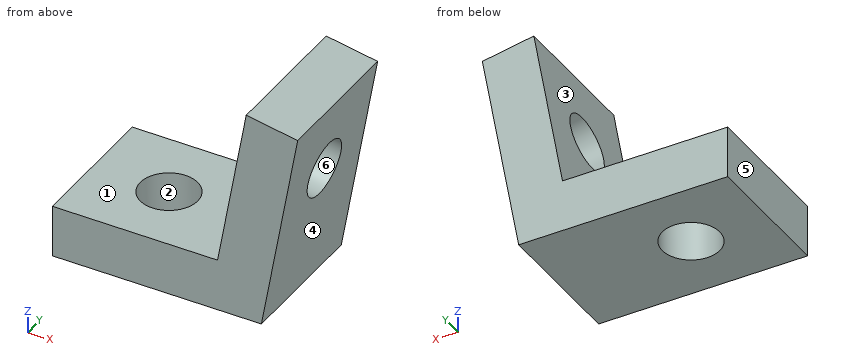
```python
from build123d import *

# Parameters (mm, degrees)
SKETCH_1_W          = 12
SKETCH_1_H          = 8
EXTRUDE_1_DEPTH     = 3
EXTRUDE_2_DEPTH     = 8
SKETCH_3_R          = 1.65
CUT_EXTRUDE_1_DEPTH = 3
SKETCH_4_R          = 1.65
CUT_EXTRUDE_2_DEPTH = 3


with BuildPart() as part:
    # 草图1 → 凸台-拉伸1 (new body)
    with BuildSketch(Plane.XY):
        with Locations((-1.4, 0)):
            Rectangle(SKETCH_1_W, SKETCH_1_H)
    extrude(amount=EXTRUDE_1_DEPTH)

    # 草图2 → 凸台-拉伸2 (add)
    with BuildSketch(Plane.XZ.offset(4)):
        Polygon((4.6, 0), (6.683778132, 11.817693036), (3.729354873, 12.338637569), (2.082701106, 3), align=None)
    extrude(amount=-EXTRUDE_2_DEPTH)

    # 草图3 → 切除-拉伸1 (cut)
    with BuildSketch(Plane.XY.offset(3)):
        with Locations((-3, 0)):
            Circle(SKETCH_3_R)
    extrude(amount=-CUT_EXTRUDE_1_DEPTH, mode=Mode.SUBTRACT)

    # 草图4 → 切除-拉伸2 (cut)
    with BuildSketch(Plane(origin=(4.461293028, 0, -0.78664633), x_dir=(-0.1736481776669236, 0, -0.9848077530122092), z_dir=(0.9848077530122092, 0, -0.1736481776669236))):
        with Locations((-8.398781617, 0)):
            Circle(SKETCH_4_R)
    extrude(amount=-CUT_EXTRUDE_2_DEPTH, mode=Mode.SUBTRACT)


solid = part.part
```
Work out the finished part from the listing and answer in its coordinate system (mm). Face numbers are marked on the shaded views. A direction names the side the tool comes from. Give positions to 0.01 mm unless a question says otherwise; leave off trailing zeros. Order: outer loops, then holes, each group sorted by start corner. A loop starts at its lowest first (then second) coordinate and runs counter-clockwise, first axis right, second up.
1. Section B-B, the plane y = -1.25 is taken. Determine the outline of the cut face in (x, z).
Result sheet:
outline: (-7.4, 0) - (-4.08, 0) - (-4.08, 3) - (-7.4, 3) - close; (-1.92, 0) - (4.6, 0) - (5.73, 6.42) - (2.78, 6.94) - (2.08, 3) - (-1.92, 3) - close; (3.15, 9.07) - (6.11, 8.55) - (6.68, 11.82) - (3.73, 12.34) - close
2. Section A-A, the plane x = -3 is taken. Determine the outline of the cut face in (y, z), and give its area (3 significant figures).
Result sheet:
outline: (-4, 0) - (-1.65, 0) - (-1.65, 3) - (-4, 3) - close; (1.65, 0) - (4, 0) - (4, 3) - (1.65, 3) - close
area: 14.1 mm2
3. Each of these flat-tipped pins is pushed along its axis until it touches: P1, Ø2.5, axis at x = -1, y = 1.5, coming from the +Z side; P2, Ø1, axis at y = 1.5, z = 4, coming from the -X side; P3, Ø4, axis at x = -1.5, y = -2, coming from the -Z side; P4, Ø4, axis at y = -0.5, z = 9.5, coming from the +X side. Where does it stop, or does it pass through?
Result sheet:
P1: stops at z = 3
P2: stops at x = 2.17
P3: stops at z = 0
P4: stops at x = 6.63
4. Section C-C, the plane z = 1.25 is taken. Determine the outline of the cut face in (x, y).
Result sheet:
outline: (-7.4, -4) - (4.82, -4) - (4.82, 4) - (-7.4, 4) - close; hole circle Ø3.3 at (-3, 0)
5. The mould has two halves that part along Z. Classify the marked faces 3, 4, 5 and 6: released by +Z, released by -Z, zero draft, split by the parting line, or undercut.
Result sheet:
face 3: released by +Z
face 4: released by -Z
face 5: zero draft
face 6: undercut
6. Section D-D, the plane x = -5.25 is taken. Determine the outline of the cut face in (y, z).
Result sheet:
outline: (-4, 0) - (4, 0) - (4, 3) - (-4, 3) - close
7. For the marked faces 1 and 2, determine the directions among +Z, -Z, +X, -X, +Y, -Y from which every point of the face is accessible in a straight line to the end or side of a thin tool.
Result sheet:
face 1: +Z, -X, +Y, -Y
face 2: +Z, -Z
8. Straight lines are drawn through the part: L1, parallel to Y at x = -3, z = 1.2; L2, parallel to Z at x = -3.25, y = 2.5; L3, parallel to X at y = 1, z = 1.5. For each, find the intervals that lie inside material, in ascending order.
Result sheet:
L1: y = -4 to -1.65, 1.65 to 4
L2: z = 0 to 3
L3: x = -7.4 to -4.31, -1.69 to 4.86
